Source: CAD feature listing. Evaluate the final solid. Frame: model axes, mm. A direction names the side the tool comes from. Give positions to 0.01 mm unless a question says otherwise; leave off trailing zeros. Order: outer loops, then holes, each group sorted by start corner. A loop starts at its lowest first (then second) coordinate and runs counter-clockwise, first axis right, second up.
from build123d import *

# Parameters (mm, degrees)
SKETCH_1_R          = 12.5
EXTRUDE_1_DEPTH     = 187
CHAMFER_1_SIZE      = 1
SKETCH_2_W          = 25
SKETCH_2_H          = 25
CUT_EXTRUDE_1_DEPTH = 2.5
SKETCH_3_R          = 5.5
CUT_EXTRUDE_2_DEPTH = 5


with BuildPart() as part:
    # 草图1 → 凸台-拉伸1 (new, symmetric)
    with BuildSketch(Plane.XY):
        Circle(SKETCH_1_R)
    extrude(amount=EXTRUDE_1_DEPTH, both=True)

    # 倒角1
    chamfer_1_edges = [part.edges().sort_by_distance(p)[0] for p in [
        (-12.5, 0, -187),
        (-12.5, 0, 187),
    ]]
    chamfer(chamfer_1_edges, length=CHAMFER_1_SIZE)

    # 草图2 → 切除-拉伸1 (cut)
    with BuildSketch(Plane(origin=(0, 12.5, 0), x_dir=(1, 0, 0), z_dir=(0, 1, 0))):
        with Locations((0, -174.5)):
            Rectangle(SKETCH_2_W, SKETCH_2_H)
        with Locations((0, 174.5)):
            Rectangle(SKETCH_2_W, SKETCH_2_H)
    cut_extrude_1 = extrude(amount=-CUT_EXTRUDE_1_DEPTH, mode=Mode.SUBTRACT)

    # 镜向1: 切除-拉伸1 across plane
    add(cut_extrude_1.mirror(Plane.ZX), mode=Mode.SUBTRACT)

    # 草图3 → 切除-拉伸2 (cut)
    with BuildSketch(Plane(origin=(12.5, 0, 0), x_dir=(0, 0, -1), z_dir=(1, 0, 0))):
        with Locations((-177.5, 0)):
            Circle(SKETCH_3_R)
        with Locations((177.5, 0)):
            Circle(SKETCH_3_R)
    extrude(amount=-CUT_EXTRUDE_2_DEPTH, mode=Mode.SUBTRACT)


solid = part.part
1) Pull-direction query (Z, two-part tool) for faces 1 (the face through (0, 10, -175)), 2 (the face through (0, 0, -187)), 3 (the face through (7.5, 0, 178)); classes: +Z half, -Z half, draft (parallel to the pull), parting line (faces both ways), or undercut.
Checks:
face 1: draft
face 2: -Z half
face 3: undercut
2) Section query B-B on z = -177.5. Output: boundary loops of the cut face in (x, y).
Checks:
outline: (-7.5, -10) - (7.5, -10) arc R12.5 ccw to (11.22, -5.5) - (7.5, -5.5) - (7.5, 5.5) - (11.22, 5.5) arc R12.5 ccw to (7.5, 10) - (-7.5, 10) arc R12.5 ccw to start
3) Section query A-A on x = 0. Output: boundary loops of the cut face in (y, z), and give its area (3 significant figures).
Checks:
outline: (-12.5, -162) - (-10, -162) - (-10, -187) - (10, -187) - (10, -162) - (12.5, -162) - (12.5, 162) - (10, 162) - (10, 187) - (-10, 187) - (-10, 162) - (-12.5, 162) - close
area: 9,100 mm2
4) Ray query, L1, parallel to X at y = -5, z = 57; L2, parallel to Z at x = 9.5, y = 3.25; L3, parallel to X at y = -1, z = -2. Return the intervals inside material, ascending.
Checks:
L1: x = -11.46 to 11.46
L2: z = -187 to -181.94, -173.06 to 173.06, 181.94 to 187
L3: x = -12.46 to 12.46
5) Section query C-C on z = 103.5. Output: boundary loops of the cut face in (x, y).
Checks:
outline: circle Ø25 at (0, 0)
6) First-contact query: pin 1 Ø3.5 at (y, z) = (2.5, 176.5) entering from +X; pin 2 Ø1 at (x, z) = (-8.5, 10.5) entering from +Y; pin 3 Ø0.8 at (x, y) = (-1.5, 11) entering from -Z. Flat tips, straight axial feed; report the tip coordinate or a pass-through.
Checks:
pin 1: stops at x = 7.5
pin 2: stops at y = 9.6
pin 3: stops at z = -162
7) Reachability of faces 4 (the face through (9.48, -2.11, -182.58)), 5 (the face through (0, -10, 174)), 6 (the face through (0, -10, -175)), 7 (the face through (0, 10, 174)) from +Z, -Z, +X, -X, +Y, -Y: full face, straight path, thin tool, end or side. Return the list, or none.
Checks:
face 4: +X
face 5: +Z, +X, -X, -Y
face 6: -Z, +X, -X, -Y
face 7: +Z, +X, -X, +Y
